For this review, take the finished solid that the model builds, in its own axes (mm). Face numbers are marked on the shaded views. A direction names the side the tool comes from. Coordinates: 2 decimals unless noted, no trailing zeros. Order: outer loops, then holes, each group sorted by start corner. A loop starts at its lowest first (then second) coordinate and runs counter-clockwise, first axis right, second up. Notation, with made-up numbers: M 0,-40 L 56,-40 A18 ccw 56,-11 Z; hole C 16.25,81 d5. An arc over 180 degrees is marked long. Use CSV: the item, a comma, the result in double quotes.
```python
from build123d import *

# Parameters (mm, degrees)
SKETCH1_R                      = 2
BOSS_EXTRUDE1_DEPTH            = 5
SKETCH2_R                      = 8.5
CUT_EXTRUDE1_DEPTH             = 2
CUT_EXTRUDE2_REACH             = 37.693
SKETCH3_R                      = 9
BOSS_EXTRUDE2_START            = 2.5
BOSS_EXTRUDE2_DEPTH            = 2.5
SKETCH5_W                      = 49
SKETCH5_H                      = 36.444930448
CUT_EXTRUDE3_DEPTH             = 11.5
F_0_8_0_8_DIAMETER_HOLE1_D     = 0.8
F_0_8_0_8_DIAMETER_HOLE1_DEPTH = 1
F_0_8_0_8_DIAMETER_HOLE1_TIP   = 0.240344248
SKETCH8_R                      = 2
BOSS_EXTRUDE3_DEPTH            = 3
F_0_8_0_8_DIAMETER_HOLE2_D     = 0.8
F_0_8_0_8_DIAMETER_HOLE2_DEPTH = 1
F_0_8_0_8_DIAMETER_HOLE2_TIP   = 0.240344248


with BuildPart() as part:
    # Sketch1 → Boss-Extrude1 (new body)
    with BuildSketch(Plane.XY):
        with BuildLine():
            Line((-26.093476939, 15), (26.093476939, 15))
            ThreePointArc((26.093476939, 15), (32, 0), (26.093476939, -15))
            Line((26.093476939, -15), (-26.093476939, -15))
            ThreePointArc((-26.093476939, -15), (-32, 0), (-26.093476939, 15))
        make_face()
        with Locations((-10, 0)):
            Circle(SKETCH1_R, mode=Mode.SUBTRACT)
        with Locations((10, 0)):
            Circle(SKETCH1_R, mode=Mode.SUBTRACT)
    extrude(amount=BOSS_EXTRUDE1_DEPTH)

    # Sketch2 → Cut-Extrude1 (cut)
    with BuildSketch(Plane(origin=(0, 0, 0), x_dir=(-1, 0, 0), z_dir=(0, 0, -1))):
        with Locations((10, 0)):
            Circle(SKETCH2_R)
    extrude(amount=-CUT_EXTRUDE1_DEPTH, mode=Mode.SUBTRACT)

    # Sketch3 → Cut-Extrude2 (cut, up to next)
    with BuildSketch(Plane(origin=(0, 0, 0), x_dir=(-1, 0, 0), z_dir=(0, 0, -1)), mode=Mode.PRIVATE) as cut_extrude2_sk1:
        with Locations((-10, 0)):
            Circle(SKETCH3_R)
    cut_extrude2_tool1 = extrude(cut_extrude2_sk1.sketch, amount=-CUT_EXTRUDE2_REACH, mode=Mode.PRIVATE) & part.part
    add(cut_extrude2_tool1.solids().sort_by_distance((10, 0, 0))[0], mode=Mode.SUBTRACT)

    # Sketch4 → Boss-Extrude2 (add)
    with BuildSketch(Plane(origin=(0, 0, 0), x_dir=(-1, 0, 0), z_dir=(0, 0, -1)).offset(BOSS_EXTRUDE2_START)):
        with BuildLine():
            ThreePointArc((26.093476939, -15), (32, 0), (26.093476939, 15))
            Line((26.093476939, 15), (23.379461873, 15))
            ThreePointArc((23.379461873, 15), (30.1, 0), (23.379461873, -15))
            Line((23.379461873, -15), (26.093476939, -15))
        make_face()
        with BuildLine():
            ThreePointArc((-26.093476939, 15), (-32, 0), (-26.093476939, -15))
            Line((-26.093476939, -15), (-23.379461873, -15))
            ThreePointArc((-23.379461873, -15), (-30.1, 0), (-23.379461873, 15))
            Line((-23.379461873, 15), (-26.093476939, 15))
        make_face()
    extrude(amount=-BOSS_EXTRUDE2_DEPTH)

    # Sketch5 → Cut-Extrude3 (cut)
    with BuildSketch(Plane(origin=(0, 0, 0), x_dir=(-1, 0, 0), z_dir=(0, 0, -1))):
        Rectangle(SKETCH5_W, SKETCH5_H)
    extrude(amount=CUT_EXTRUDE3_DEPTH, mode=Mode.SUBTRACT)

    # Ø0.8 (0.8) Diameter Hole1
    with Locations(Plane(origin=(1, 12.5, 0), x_dir=(-1, 0, 0), z_dir=(0, 0, -1))):
        with Locations((0, 0), (-20, 0)):
            Hole(F_0_8_0_8_DIAMETER_HOLE1_D / 2, depth=F_0_8_0_8_DIAMETER_HOLE1_DEPTH)
            with Locations((0, 0, -(F_0_8_0_8_DIAMETER_HOLE1_DEPTH + F_0_8_0_8_DIAMETER_HOLE1_TIP / 2))):  # 118° drill point
                Cone(0, F_0_8_0_8_DIAMETER_HOLE1_D / 2, F_0_8_0_8_DIAMETER_HOLE1_TIP, mode=Mode.SUBTRACT)

    # Sketch8 → Boss-Extrude3 (add)
    with BuildSketch(Plane(origin=(0, 0, 2), x_dir=(-1, 0, 0), z_dir=(0, 0, -1))):
        with Locations((10, 0)):
            Circle(SKETCH8_R)
    extrude(amount=-BOSS_EXTRUDE3_DEPTH)

    # Ø0.8 (0.8) Diameter Hole2
    with Locations(Plane(origin=(-16, 15, 2.8), x_dir=(1, 0, 0), z_dir=(0, 1, 0))):
        with Locations((0, 0), (20, 0)):
            Hole(F_0_8_0_8_DIAMETER_HOLE2_D / 2, depth=F_0_8_0_8_DIAMETER_HOLE2_DEPTH)
            with Locations((0, 0, -(F_0_8_0_8_DIAMETER_HOLE2_DEPTH + F_0_8_0_8_DIAMETER_HOLE2_TIP / 2))):  # 118° drill point
                Cone(0, F_0_8_0_8_DIAMETER_HOLE2_D / 2, F_0_8_0_8_DIAMETER_HOLE2_TIP, mode=Mode.SUBTRACT)


solid = part.part
```
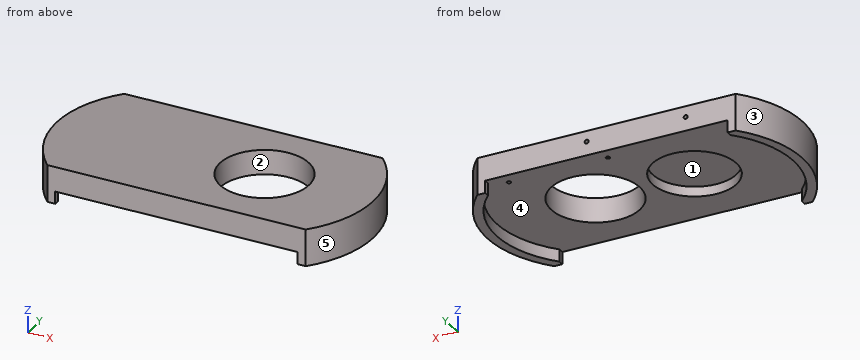
Item 1: To check wall thickness, follow line 1 along Z through (x, y) = (4, 14); line 2 along X through (y, z) = (14.65, 2.8); line 3 along X through (y, z) = (6.5, 0.25). State the ranges of each line that lie inside material, in increasing order. Write a range as [from, to].
Solutions:
line 1,"[0, 2.4], [3.2, 5]"
line 2,"[-26.41, -16.4], [-15.6, 3.6], [4.4, 26.41]"
line 3,"[-31.02, -15.48], [-4.52, 3.78], [16.22, 31.02]"
Item 2: Draft analysis for pull direction X (two halves, no side actions). For the marked faces 3, 4 and 5, state which applies: released by +X, released by -X, zero draft, split by the parting line, or undercut.
Solutions:
face 3,"released by -X"
face 4,"undercut"
face 5,"released by +X"
Item 3: Add section D-D on y = 0. State the section outline as (x, z) points, and give its area (4 significant figures).
Solutions:
outline,"M -32,-2.5 L -30.1,-2.5 L -30.1,0 L -18.5,0 L -18.5,2 L -1.5,2 L -1.5,0 L 1,0 L 1,5 L -32,5 Z; M 19,0 L 30.1,0 L 30.1,-2.5 L 32,-2.5 L 32,5 L 19,5 Z"
area,"205.5 mm^2"
Item 4: For the marked faces 1 and 2, list the 3-axis set-ups (+Z, -Z, +X, -X, +Y, -Y) from which the entire face can be reached by the end or side of a thin tool; tool diameter is ignored.
Solutions:
face 1,"-Z"
face 2,"+Z, -Z"
Item 5: Clearance check with flat-ended pins moving along their axes: pin 1 Ø8.5 at (x, y) = (-13, 0.5) entering from -Z; pin 2 Ø0.9 at (y, z) = (14.5, -1) entering from +X; pin 3 Ø0.9 at (y, z) = (-14, -1) entering from -X. State where each tip first meets the part, or that it passes through.
Solutions:
pin 1,"z = 2"
pin 2,"x = 26.93"
pin 3,"x = -27.33"
Item 6: Add section B-B on x = 10. State the section outline as (y, z) points, and give its area (3 significant figures).
Solutions:
outline,"M -15,0 L -9,0 L -9,5 L -15,5 Z; M 9,0 L 15,0 L 15,5 L 9,5 Z"
area,"60.0 mm^2"
Item 7: Add section C-C on y = -4. State the section outline as (x, z) points.
Solutions:
outline,"M -31.63,-2.5 L -29.7,-2.5 L -29.7,0 L -17.5,0 L -17.5,2 L -2.5,2 L -2.5,0 L 1.94,0 L 1.94,5 L -31.63,5 Z; M 18.06,0 L 29.7,0 L 29.7,-2.5 L 31.63,-2.5 L 31.63,5 L 18.06,5 Z"
Item 8: Add section A-A on z = -1. State the section outline as (x, y) points, and give its area (3 significant figures).
Solutions:
outline,"M -26.09,-15 L -24.5,-15 L -24.5,-13.92 A20.1 cw -24.5,13.92 L -24.5,15 L -26.09,15 A22 ccw Z; M 24.5,-15 L 26.09,-15 A22 ccw 26.09,15 L 24.5,15 L 24.5,13.92 A20.1 cw 24.5,-13.92 Z"
area,"125 mm^2"
